Work out the finished part from the listing and answer in its coordinate system (mm). Coordinates: 2 decimals unless noted, no trailing zeros. Write each loop counter-clockwise with the first axis right and the second up, starting at its lowest first coordinate (ties: lowest second). Pieces come first, ordered by that corner, then holes. Notation, with made-up numbers: (27, 40) -> (76, 40) arc R12 cw to (76, 59) -> close; hole circle Ø5 at (43, -4). An arc over 180 degrees is marked (long way). Write each question's results on one line, items separated by ' | '. Start each with the question number.
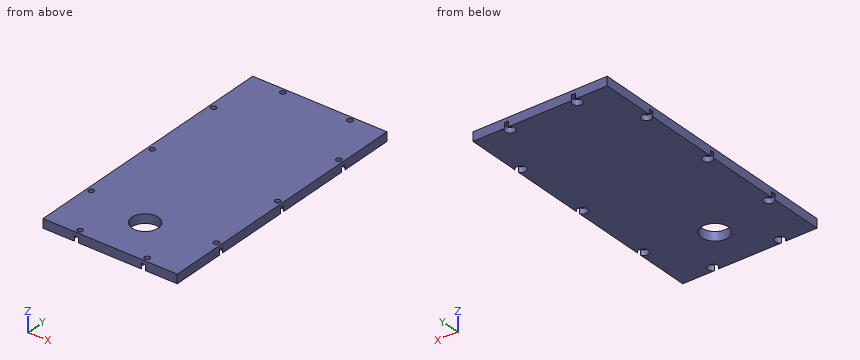
from build123d import *

# Parameters (mm, degrees)
SKETCH_1_W                   = 60
SKETCH_1_H                   = 120
EXTRUDE_1_DEPTH              = 2
HOLE_WIZARD_M2_1_D           = 2.4
HOLE_WIZARD_M2_1_CBORE_D     = 4.4
HOLE_WIZARD_M2_1_CBORE_DEPTH = 2.4
SKETCH_7_R                   = 5.9
CUT_EXTRUDE_2_DEPTH          = 68.201190466


with BuildPart() as part:
    # 草图1 → 凸台-拉伸1 (new, symmetric)
    with BuildSketch(Plane.XY):
        Rectangle(SKETCH_1_W, SKETCH_1_H)
    extrude(amount=EXTRUDE_1_DEPTH, both=True)

    # M2 六角凹头螺钉的柱形沉头孔1 (through all)
    with Locations(Plane(origin=(0, 0, -2), x_dir=(-1, 0, 0), z_dir=(0, 0, -1))):
        with Locations((-15, -58), (-28, 0), (28, 0), (-15, 58), (15, 58), (-28, 35), (28, 35), (-28, -35), (28, -35), (15, -58)):
            CounterBoreHole(HOLE_WIZARD_M2_1_D / 2, HOLE_WIZARD_M2_1_CBORE_D / 2, HOLE_WIZARD_M2_1_CBORE_DEPTH)

    # 草图7 → 切除-拉伸2 (cut, through all)
    with BuildSketch(Plane(origin=(0, 0, -2), x_dir=(-1, 0, 0), z_dir=(0, 0, -1))):
        with Locations((0, -40)):
            Circle(SKETCH_7_R)
    extrude(amount=-CUT_EXTRUDE_2_DEPTH, mode=Mode.SUBTRACT)


solid = part.part
1. Find section A-A on x = 0. Give the vertices of the cut face in (y, z), and give its area (3 significant figures).
2. Find the intervals of material crossed by L1, parallel to Y at x = 15, z = 0.8; L2, parallel to Y at x = -28, z = 1.45; L3, parallel to Y at x = -13.5, z = 0.1, in increasing order.
3. Find section D-D on z = -1.2. Give the vertices of the cut face in (x, y), and give its area (3 significant figures).
4. Find section C-C on x = 28. Give the vertices of the cut face in (y, z).
5. Given pin 1 Ø2 at (x, y) = (-28, -35) entering from -Z; pin 2 Ø3 at (x, y) = (-15, 58) entering from -Z, each flat-ended and moving along its own axis, determine where each tip first touches the part or whether it passes through.
6. Find section B-B on y = -40. Give the vertices of the cut face in (x, z), and give its area (3 significant figures).
Ans:
1) outline: (-60, -2) -> (-45.9, -2) -> (-45.9, 2) -> (-60, 2) -> close; (-34.1, -2) -> (60, -2) -> (60, 2) -> (-34.1, 2) -> close | area: 433 mm²
2) L1: y = -60 to -59.2, -56.8 to 56.8, 59.2 to 60 | L2: y = -60 to -36.2, -33.8 to -1.2, 1.2 to 33.8, 36.2 to 60 | L3: y = -60 to -59.61, -56.39 to 56.39, 59.61 to 60
3) outline: (-30, -60) -> (-15.92, -60) arc R2.2 cw (long way) to (-14.08, -60) -> (14.08, -60) arc R2.2 cw (long way) to (15.92, -60) -> (30, -60) -> (30, -35.92) arc R2.2 cw (long way) to (30, -34.08) -> (30, -0.92) arc R2.2 cw (long way) to (30, 0.92) -> (30, 34.08) arc R2.2 cw (long way) to (30, 35.92) -> (30, 60) -> (15.92, 60) arc R2.2 cw (long way) to (14.08, 60) -> (-14.08, 60) arc R2.2 cw (long way) to (-15.92, 60) -> (-30, 60) -> (-30, 35.92) arc R2.2 cw (long way) to (-30, 34.08) -> (-30, 0.92) arc R2.2 cw (long way) to (-30, -0.92) -> (-30, -34.08) arc R2.2 cw (long way) to (-30, -35.92) -> close; hole circle Ø11.8 at (0, -40) | area: 6,940 mm²
4) outline: (-60, -2) -> (-37.2, -2) -> (-37.2, 0.4) -> (-36.2, 0.4) -> (-36.2, 2) -> (-60, 2) -> close; (-33.8, 0.4) -> (-32.8, 0.4) -> (-32.8, -2) -> (-2.2, -2) -> (-2.2, 0.4) -> (-1.2, 0.4) -> (-1.2, 2) -> (-33.8, 2) -> close; (1.2, 0.4) -> (2.2, 0.4) -> (2.2, -2) -> (32.8, -2) -> (32.8, 0.4) -> (33.8, 0.4) -> (33.8, 2) -> (1.2, 2) -> close; (36.2, 0.4) -> (37.2, 0.4) -> (37.2, -2) -> (60, -2) -> (60, 2) -> (36.2, 2) -> close
5) pin 1: passes through | pin 2: stops at z = 0.4
6) outline: (-30, -2) -> (-5.9, -2) -> (-5.9, 2) -> (-30, 2) -> close; (5.9, -2) -> (30, -2) -> (30, 2) -> (5.9, 2) -> close | area: 193 mm²
